Here's how the part is built. I have some questions about the finished solid (model axes, mm). Face numbers are marked on the shaded views. A direction names the side the tool comes from. Give positions to 0.01 mm unless a question says otherwise; leave off trailing zeros. Loops run counter-clockwise (first coordinate to the right, second up) from the corner with the lowest first, then second, coordinate; pieces in that order, holes last.
Q1. Thinking about a two-plate mould opening in X: for the marked faces 4, 5 and 6, which applies, pulls with the +X half, pulls with the -X half, needs draft (parallel to the pull), parting line crosses it, or undercut?
Q2. Suppose I cut it at C-C (z = 21.5). List the corners of the cut face in (x, y) for me.
Q3. I'm going to push flat-ended pins straight in: P1, Ø2, axis at y = 29, z = 14, coming from the +X side; P2, Ø4, axis at y = -38.5, z = 12, coming from the -X side; P3, Ø12, axis at x = -9, z = 33.5, coming from the +Y side. Where does each tip first touch, or does it pass through?
Q4. I need wall thicknesses on probe 1 along Y at (x, z) = (0, 17); probe 2 along X at (y, z) = (11, 34); probe 3 along Z at (x, y) = (33.5, 11.5). Which ranges of each line are inside material? Lowest first, please.
Q5. Suppose I cut it at A-A (x = -9). List the corners of the cut face in (y, z) for me, and give its area (3 significant figures).
Q6. Suppose I cut it at D-D (x = -22). List the corners of the cut face in (y, z) for me, and give its area (3 significant figures).
Q7. Suppose I cut it at B-B (y = 0). List the corners of the cut face in (x, z) for me, and give its area (3 significant figures).
Q8. For the marked faces 1, 2 and 3, which set-ups out of +Z, -Z, +X, -X, +Y, -Y let a thin tool reach every point of the face, with its end or its side?
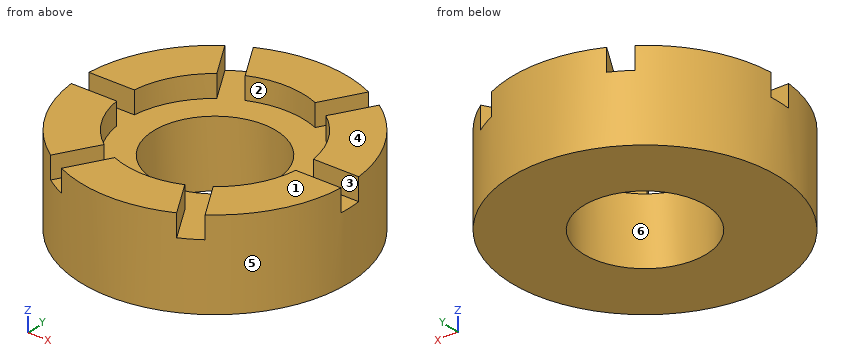
```python
from build123d import *

# Parameters (mm, degrees)
SKETCH_1_R               = 60
EXTRUDE_1_DEPTH          = 40
SKETCH_2_R               = 40
CUT_EXTRUDE_1_DEPTH      = 10
CUT_EXTRUDE_2_REACH      = 92
SKETCH_3_R               = 27.5
SKETCH_4_W               = 150
SKETCH_4_H               = 10
CUT_EXTRUDE_3_DEPTH      = 10
PATTERN_CIRCULAR_1_COUNT = 3


with BuildPart() as part:
    # 草图1 → 凸台-拉伸1 (new body)
    with BuildSketch(Plane.XY):
        Circle(SKETCH_1_R)
    extrude(amount=EXTRUDE_1_DEPTH)

    # 草图2 → 切除-拉伸1 (cut)
    with BuildSketch(Plane.XY.offset(40)):
        Circle(SKETCH_2_R)
    extrude(amount=-CUT_EXTRUDE_1_DEPTH, mode=Mode.SUBTRACT)

    # 草图3 → 切除-拉伸2 (cut, up to next)
    with BuildSketch(Plane.XY.offset(30), mode=Mode.PRIVATE) as cut_extrude_2_sk1:
        Circle(SKETCH_3_R)
    cut_extrude_2_tool1 = extrude(cut_extrude_2_sk1.sketch, amount=-CUT_EXTRUDE_2_REACH, mode=Mode.PRIVATE) & part.part
    add(cut_extrude_2_tool1.solids().sort_by_distance((0, 0, 30))[0], mode=Mode.SUBTRACT)

    # 草图4 → 切除-拉伸3 (cut)
    with BuildSketch(Plane.XY.offset(30)):
        Rectangle(SKETCH_4_W, SKETCH_4_H)
    cut_extrude_3 = extrude(amount=CUT_EXTRUDE_3_DEPTH, mode=Mode.SUBTRACT)

    # 阵列(圆周)1: 切除-拉伸3 ×3 about axis
    pattern_circular_1_axis = Axis((0, 0, 0), (0, 0, 1))
    for i in range(1, PATTERN_CIRCULAR_1_COUNT):
        add(cut_extrude_3.rotate(pattern_circular_1_axis, i * 360 / PATTERN_CIRCULAR_1_COUNT), mode=Mode.SUBTRACT)


solid = part.part
```
Solutions:
1. face 4: needs draft
1. face 5: parting line crosses it
1. face 6: undercut
2. outline: circle Ø120 at (0, 0); hole circle Ø55 at (0, 0)
3. P1: stops at x = 53.07
3. P2: stops at x = -47.62
3. P3: stops at y = 59.92
4. probe 1: y = -60 to -27.5, 27.5 to 60
4. probe 2: x = -58.98 to -38.46, 38.46 to 58.98
4. probe 3: z = 0 to 30
5. outline: (-59.32, 0) - (-25.99, 0) - (-25.99, 30) - (-38.97, 30) - (-38.97, 40) - (-59.32, 40) - close; (25.99, 0) - (59.32, 0) - (59.32, 40) - (38.97, 40) - (38.97, 30) - (25.99, 30) - close
5. area: 2,410 mm2
6. outline: (-55.82, 0) - (-16.5, 0) - (-16.5, 30) - (-48.11, 30) - (-48.11, 40) - (-55.82, 40) - close; (16.5, 0) - (55.82, 0) - (55.82, 40) - (48.11, 40) - (48.11, 30) - (16.5, 30) - close
6. area: 2,510 mm2
7. outline: (-60, 0) - (-27.5, 0) - (-27.5, 30) - (-60, 30) - close; (27.5, 0) - (60, 0) - (60, 30) - (27.5, 30) - close
7. area: 1,950 mm2
8. face 1: +Z, +X, -X, +Y, -Y
8. face 2: +Z
8. face 3: +Z, +X, -X
